Can you work these out from the model? Positions are in its coordinate system, mm. A direction names the side the tool comes from. Give positions to 0.01 mm unless a question says otherwise; leave off trailing zeros. Order: outer loops, then holes, each group sorted by start corner. A loop starts at its lowest first (then second) coordinate and runs counter-clockwise, first axis right, second up. Notation, with made-up numbers: (12, 78.25) - (51, 78.25) arc R30 ccw to (51, 106.25) - close; hole circle Ø3 at (68.5, 14.25). An arc over 180 degrees is marked (long way). Use one line per item in the form item = value. Start each with the question number.
1) Suppose I cut it at A-A, the plane y = 34. Write out the boundary of the cut face in (x, z), and give its area (3 significant figures).
2) Suppose I cut it at D-D, the plane x = -66.5. Write out the boundary of the cut face in (y, z).
3) We'd pull the mould along Y, two halves only. Please class faces 1 (the conical face through (-0.339, 25.531, 47.526)), 2 (the cylindrical face through (-55, 47, 14)), 3 (the flat face through (-1, 12, 77)): released by +Y, released by -Y, zero draft, split by the parting line, or undercut.
4) Suppose I cut it at B-B, the plane z = 0. Write out the boundary of the cut face in (x, y).
5) Which directions (+Z, -Z, +X, -X, +Y, -Y) give clear straight access to the entire face, cutting with the end or side of a thin tool? Please do faces 4 (the flat face through (-21.927, 40.283, -35.268)), 5 (the flat face through (-63, 34, -14)), 6 (the flat face through (-47, 40, 9)), 7 (the cylindrical face through (1.172, 42.313, 37.077)).
6) For pin 1 (8 mm diameter, centred on y = 33.5, z = 15, fed in from -X); pin 2 (4 mm diameter, centred on y = 5.5, z = -61, fed in from -X); pin 3 (14.5 mm diameter, centred on y = 40.5, z = -1.5, fed in from +X), each with a flat end and sliding along its axis, tell me the tip position at first contact or that it passes through.
7) Suppose I cut it at C-C, the plane z = -24. Write out the boundary of the cut face in (x, y), and give its area (3 significant figures).
8) Please list where these lines run through material, in increasing order: probe 1 along X at (y, z) = (16.75, -51); probe 2 along Z at (x, y) = (3, 50.5); probe 3 along Y at (x, z) = (51, 16).
```python
from build123d import *

# Parameters (mm, degrees)
BASE_PLATE_154X154X25_DEPTH      = 25
LOCATING_SPIGOT_SKETCH_112_R     = 56
LOCATING_SPIGOT_112X6_DEPTH      = 6
PIVOT_BOSS_WITH_LUGS_DEPTH       = 31
PIVOT_BOSS_FILLETS_R12_R         = 12
LUG_PIN_HOLES_SKETCH_10_R        = 5
LUG_PIN_HOLES_10_DEPTH           = 136.207248326
CENTRE_BORE_SKETCH_40_R          = 20
CENTRE_BORE_40_DEPTH             = 42
THROUGH_BORE_SKETCH_28_R         = 14
THROUGH_BORE_28_DEPTH            = 42
TAPPED_HOLES_M20X2_0_D           = 18
TAPPED_HOLES_M20X2_0_DEPTH       = 26
TAPPED_HOLES_M20X2_0_CSINK_D     = 20.05
TAPPED_HOLES_M20X2_0_CSINK_ANGLE = 90
TAPPED_HOLES_M20X2_0_TIP         = 5.407745571
MOUNTING_HOLES_SKETCH_4X_20_R    = 10
MOUNTING_HOLES_4X_20_DEPTH       = 42


with BuildPart() as part:
    # Base Plate Profile 154x154 R26 → Base Plate 154x154x25 (new body)
    with BuildSketch(Plane(origin=(0, 0, 0), x_dir=(1, 0, 0), z_dir=(0, 1, 0))):
        with BuildLine():
            Line((-51, -77), (51, -77))
            ThreePointArc((51, -77), (69.384776311, -69.384776311), (77, -51))
            Line((77, -51), (77, 51))
            ThreePointArc((77, 51), (69.384776311, 69.384776311), (51, 77))
            Line((51, 77), (-51, 77))
            ThreePointArc((-51, 77), (-69.384776311, 69.384776311), (-77, 51))
            Line((-77, 51), (-77, -51))
            ThreePointArc((-77, -51), (-69.384776311, -69.384776311), (-51, -77))
        make_face()
    extrude(amount=BASE_PLATE_154X154X25_DEPTH)

    # Locating Spigot Sketch Ø112 → Locating Spigot Ø112x6 (add)
    with BuildSketch(Plane.XZ):
        with Locations(Location((0, 0, 0), (0, 0, 270))):
            Circle(LOCATING_SPIGOT_SKETCH_112_R)
    extrude(amount=LOCATING_SPIGOT_112X6_DEPTH)

    # Pivot Boss Profile → Pivot Boss with Lugs (add)
    with BuildSketch(Plane(origin=(0, 25, 0), x_dir=(1, 0, 0), z_dir=(0, 1, 0))):
        with BuildLine():
            Line((-17.266235066, 51.086956522), (-26.719653956, 19))
            Line((-26.719653956, 19), (-63, 19))
            Line((-63, 19), (-63, 9))
            Line((-63, 9), (-31, 9))
            Line((-31, 9), (-31, -9))
            Line((-31, -9), (-63, -9))
            Line((-63, -9), (-63, -19))
            Line((-63, -19), (-26.719653956, -19))
            Line((-26.719653956, -19), (-17.266235066, -51.086956522))
            ThreePointArc((-17.266235066, -51.086956522), (0, -64), (17.266235066, -51.086956522))
            Line((17.266235066, -51.086956522), (26.719653956, -19))
            Line((26.719653956, -19), (63, -19))
            Line((63, -19), (63, -9))
            Line((63, -9), (31, -9))
            Line((31, -9), (31, 9))
            Line((31, 9), (63, 9))
            Line((63, 9), (63, 19))
            Line((63, 19), (26.719653956, 19))
            Line((26.719653956, 19), (17.266235066, 51.086956522))
            ThreePointArc((17.266235066, 51.086956522), (0, 64), (-17.266235066, 51.086956522))
        make_face()
    extrude(amount=PIVOT_BOSS_WITH_LUGS_DEPTH)

    # Pivot Boss Fillets R12
    pivot_boss_fillets_r12_edges = [part.edges().sort_by_distance(p)[0] for p in [
        (-63, 56, 14),
        (63, 56, 14),
        (63, 56, -14),
        (-63, 56, -14),
    ]]
    fillet(pivot_boss_fillets_r12_edges, radius=PIVOT_BOSS_FILLETS_R12_R)

    # Lug Pin Holes Sketch Ø10 → Lug Pin Holes Ø10 (cut, through all)
    with BuildSketch(Plane.XY.offset(19)):
        with Locations((-51, 44)):
            Circle(LUG_PIN_HOLES_SKETCH_10_R)
        with Locations((51, 44)):
            Circle(LUG_PIN_HOLES_SKETCH_10_R)
    extrude(amount=-LUG_PIN_HOLES_10_DEPTH, mode=Mode.SUBTRACT)

    # Centre Bore Sketch Ø40 → Centre Bore Ø40 (cut)
    with BuildSketch(Plane(origin=(0, 56, 0), x_dir=(1, 0, 0), z_dir=(0, 1, 0))):
        with Locations(Location((0, 0, 0), (0, 0, 270))):
            Circle(CENTRE_BORE_SKETCH_40_R)
    extrude(amount=-CENTRE_BORE_40_DEPTH, mode=Mode.SUBTRACT)

    # Through Bore Sketch Ø28 → Through Bore Ø28 (cut)
    with BuildSketch(Plane(origin=(0, 14, 0), x_dir=(1, 0, 0), z_dir=(0, 1, 0))):
        with Locations(Location((0, 0, 0), (0, 0, 270))):
            Circle(THROUGH_BORE_SKETCH_28_R)
    extrude(amount=-THROUGH_BORE_28_DEPTH, mode=Mode.SUBTRACT)

    # Tapped Holes M20x2.0
    with Locations(Plane(origin=(0, 56, 0), x_dir=(1, 0, 0), z_dir=(0, 1, 0))):
        with Locations((0, 46), (0, -46)):
            CounterSinkHole(TAPPED_HOLES_M20X2_0_D / 2, TAPPED_HOLES_M20X2_0_CSINK_D / 2, depth=TAPPED_HOLES_M20X2_0_DEPTH, counter_sink_angle=TAPPED_HOLES_M20X2_0_CSINK_ANGLE)
            with Locations((0, 0, -(TAPPED_HOLES_M20X2_0_DEPTH + TAPPED_HOLES_M20X2_0_TIP / 2))):  # 118° drill point
                Cone(0, TAPPED_HOLES_M20X2_0_D / 2, TAPPED_HOLES_M20X2_0_TIP, mode=Mode.SUBTRACT)

    # Mounting Holes Sketch 4xØ20 → Mounting Holes 4xØ20 (cut)
    with BuildSketch(Plane(origin=(0, 25, 0), x_dir=(1, 0, 0), z_dir=(0, 1, 0))):
        with Locations(Location((51, 51, 0), (0, 0, 270))):
            Circle(MOUNTING_HOLES_SKETCH_4X_20_R)
        with Locations(Location((-51, 51, 0), (0, 0, 270))):
            Circle(MOUNTING_HOLES_SKETCH_4X_20_R)
        with Locations(Location((-51, -51, 0), (0, 0, 270))):
            Circle(MOUNTING_HOLES_SKETCH_4X_20_R)
        with Locations(Location((51, -51, 0), (0, 0, 270))):
            Circle(MOUNTING_HOLES_SKETCH_4X_20_R)
    extrude(amount=-MOUNTING_HOLES_4X_20_DEPTH, mode=Mode.SUBTRACT)


solid = part.part
```
Result sheet:
q1.outline = (-63, -19) - (-26.72, -19) - (-17.27, -51.09) arc R18 ccw to (17.27, -51.09) - (26.72, -19) - (63, -19) - (63, -9) - (31, -9) - (31, 9) - (63, 9) - (63, 19) - (26.72, 19) - (17.27, 51.09) arc R18 ccw to (-17.27, 51.09) - (-26.72, 19) - (-63, 19) - (-63, 9) - (-31, 9) - (-31, -9) - (-63, -9) - close; hole circle Ø40 at (0, 0); hole circle Ø18 at (0, -46); hole circle Ø18 at (0, 46)
q1.area = 5,350 mm²
q2.outline = (0, -71.87) - (25, -71.87) - (25, 71.87) - (0, 71.87) - close
q3.face_1 = released by +Y
q3.face_2 = undercut
q3.face_3 = zero draft
q4.outline = (-77, 0) - (-56, 0) - (-56, -6) - (-14, -6) - (-14, 14) - (-20, 14) - (-20, 56) - (-31, 56) - (-31, 25) - (-77, 25) - close; (14, -6) - (56, -6) - (56, 0) - (77, 0) - (77, 25) - (31, 25) - (31, 56) - (20, 56) - (20, 14) - (14, 14) - close
q5.face_4 = -Z, -X, +Y
q5.face_5 = +Z, -Z, -X, +Y
q5.face_6 = -X, +Y
q5.face_7 = +Y
q6.pin_1 = -63
q6.pin_2 = -75.74
q6.pin_3 = 31
q7.outline = (-77, 0) - (-50.6, 0) - (-50.6, -6) - (50.6, -6) - (50.6, 0) - (77, 0) - (77, 25) - (25.25, 25) - (25.25, 56) - (-25.25, 56) - (-25.25, 25) - (-77, 25) - close
q7.area = 6,020 mm²
q8.probe_1 = -77 to -61, -41 to 41, 61 to 77
q8.probe_2 = -63.75 to -54.49, -37.51 to -19.77, 19.77 to 37.51, 54.49 to 63.75
q8.probe_3 = -6 to 39, 49 to 56
